Build history of the part. All positions in model axes, mm. Face numbers are marked on the shaded views. A direction names the side the tool comes from. Round coordinates to 2 decimals unless told otherwise and drop trailing zeros. Loops run counter-clockwise (first coordinate to the right, second up) from the corner with the lowest first, then second, coordinate; pieces in that order, holes last. Notation, with made-up numbers: (58, 23.5) - (80, 23.5) arc R4 cw to (80, 30.5) - close; hole circle Ø3 at (24, 23). An arc over 180 degrees is marked (long way). Use a Markdown table: item, result.
from build123d import *

# Parameters (mm, degrees)
BASE_BLOCK_SKETCH_W       = 90
BASE_BLOCK_SKETCH_H       = 45
BASE_BLOCK_90X45X60_DEPTH = 60
LUG_A_SKETCH_R            = 10
LUG_A_DEPTH               = 20
LUG_RECESS_CUT_DEPTH      = 5
LUG_B_DEPTH               = 20
LUG_HOLE_SKETCH_R         = 10
LUG_HOLES_DEPTH           = 114.357840488
ANGLED_SIDE_CUT_SKETCH_W  = 35
ANGLED_SIDE_CUT_SKETCH_H  = 40
ANGLED_SIDE_CUT_DEPTH     = 117.216392992
SIDE_BOSS_A_SKETCH_R      = 7.5
SIDE_BOSS_A_DEPTH         = 20
SIDE_BOSS_B_SKETCH_R      = 7.5
SIDE_BOSS_B_DEPTH         = 20
TOP_HOLE_SKETCH_R         = 12.5
TOP_HOLE_DEPTH            = 20
LUG_TOP_FILLET_R18_R      = 18
BOTTOM_SLOT_SKETCH_W      = 10
BOTTOM_SLOT_SKETCH_H      = 40
BOTTOM_SLOT_DEPTH         = 129.570019834


with BuildPart() as part:
    # Base Block Sketch → Base Block 90x45x60 (new body)
    with BuildSketch(Plane(origin=(0, 0, 0), x_dir=(1, 0, 0), z_dir=(0, 1, 0))):
        Rectangle(BASE_BLOCK_SKETCH_W, BASE_BLOCK_SKETCH_H)
    extrude(amount=-BASE_BLOCK_90X45X60_DEPTH)

    # Lug A Sketch → Lug A (add)
    with BuildSketch(Plane.XY.offset(22.5)):
        Polygon((-45, 0), (-45, -60), (45, -60), (45, 0), (0, 40), (-45, 40), align=None)
        with Locations((-8, 20)):
            Circle(LUG_A_SKETCH_R, mode=Mode.SUBTRACT)
    extrude(amount=LUG_A_DEPTH)

    # Lug Recess Sketch → Lug Recess Cut (cut)
    with BuildSketch(Plane(origin=(0, 0, 22.5), x_dir=(-1, 0, 0), z_dir=(0, 0, -1))):
        Polygon((-45, 0), (45, 0), (45, 40), (0, 40), align=None)
    extrude(amount=-LUG_RECESS_CUT_DEPTH, mode=Mode.SUBTRACT)

    # Lug B Sketch → Lug B (add)
    with BuildSketch(Plane(origin=(0, 0, -22.5), x_dir=(-1, 0, 0), z_dir=(0, 0, -1))):
        Polygon((-45, 0), (-45, -60), (45, -60), (45, 0), (45, 40), (0, 40), align=None)
    extrude(amount=LUG_B_DEPTH)

    # Lug Hole Sketch → Lug Holes (cut, through all)
    with BuildSketch(Plane.XY.offset(42.5)):
        with Locations((-8, 20)):
            Circle(LUG_HOLE_SKETCH_R)
    extrude(amount=-LUG_HOLES_DEPTH, mode=Mode.SUBTRACT)

    # Angled Side Cut Sketch → Angled Side Cut (cut, through all)
    with BuildSketch(Plane(origin=(45, 0, 0), x_dir=(0, 0, -1), z_dir=(1, 0, 0))):
        with Locations((-5, -40)):
            Rectangle(ANGLED_SIDE_CUT_SKETCH_W, ANGLED_SIDE_CUT_SKETCH_H)
    extrude(amount=-ANGLED_SIDE_CUT_DEPTH, mode=Mode.SUBTRACT)

    # Side Boss A Sketch → Side Boss A (add)
    with BuildSketch(Plane.ZY.offset(45)):
        with BuildLine():
            ThreePointArc((68.287962614, -7.064659931), (67.675104993, 4.552186853), (57.5, 10.190800338))
            Line((57.5, 10.190800338), (42.5, 10.190800338))
            Line((42.5, 10.190800338), (42.5, -60))
            Line((42.5, -60), (68.287962614, -7.064659931))
        make_face()
        with Locations((57.5, -1.809199662)):
            Circle(SIDE_BOSS_A_SKETCH_R, mode=Mode.SUBTRACT)
    extrude(amount=-SIDE_BOSS_A_DEPTH)

    # Side Boss B Sketch → Side Boss B (add)
    with BuildSketch(Plane.ZY.offset(45)):
        with BuildLine():
            Line((-42.5, 12), (-57.5, 12))
            ThreePointArc((-57.5, 12), (-67.633293922, 6.427779888), (-68.355763811, -5.113940953))
            Line((-68.355763811, -5.113940953), (-42.5, -60))
            Line((-42.5, -60), (-42.5, 12))
        make_face()
        with Locations((-57.5, 0)):
            Circle(SIDE_BOSS_B_SKETCH_R, mode=Mode.SUBTRACT)
    extrude(amount=-SIDE_BOSS_B_DEPTH)

    # Top Hole Sketch → Top Hole (cut)
    with BuildSketch(Plane(origin=(0, 0, 0), x_dir=(1, 0, 0), z_dir=(0, 1, 0))):
        with Locations(Location((30, -2.5, 0), (0, 0, 270))):
            Circle(TOP_HOLE_SKETCH_R)
    extrude(amount=-TOP_HOLE_DEPTH, mode=Mode.SUBTRACT)

    # Lug Top Fillet R18
    lug_top_fillet_r18_edges = [part.edges().sort_by_distance(p)[0] for p in [
        (0, 40, 35),
        (0, 40, -32.5),
    ]]
    fillet(lug_top_fillet_r18_edges, radius=LUG_TOP_FILLET_R18_R)

    # Bottom Slot Sketch → Bottom Slot (cut, through all)
    with BuildSketch(Plane(origin=(45, 0, 0), x_dir=(0, 0, -1), z_dir=(1, 0, 0))):
        with Locations((17.5, -40)):
            Rectangle(BOTTOM_SLOT_SKETCH_W, BOTTOM_SLOT_SKETCH_H)
    extrude(amount=-BOTTOM_SLOT_DEPTH, mode=Mode.SUBTRACT)


solid = part.part
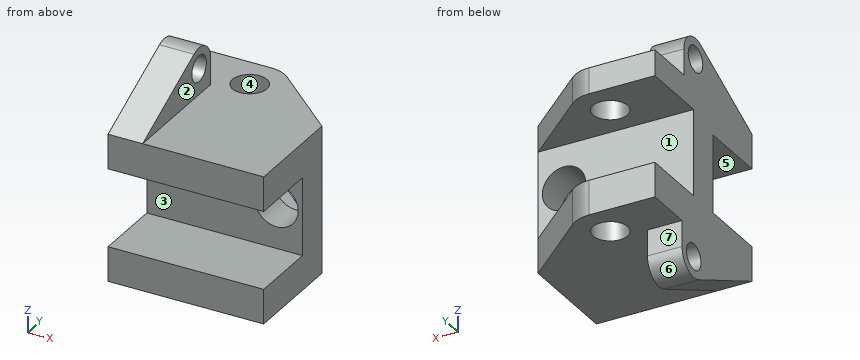
Q1. Cut at C-C, the plane x = 30. List the corners of the cut face in (y, z), plus the area to 3 significant figures.
Results found:
| item | result |
|---|---|
| outline | (-60, -42.5) - (13.33, -42.5) - (13.33, -22.5) - (0, -22.5) - (0, -10) - (-20, -10) - (-20, -22.5) - (-60, -22.5) - close; (-60, 22.5) - (-20, 22.5) - (-20, 15) - (0, 15) - (0, 27.5) - (13.33, 27.5) - (13.33, 42.5) - (-60, 42.5) - close |
| area | 3,270 mm2 |
Q2. Cut at A-A, the plane x = -16. List the corners of the cut face in (y, z), plus the area to 3 significant figures.
Results found:
| item | result |
|---|---|
| outline | (-60, -42.5) - (14, -42.5) - (14, -22.5) - (0, -22.5) - (0, 27.5) - (14, 27.5) - (14, 42.5) - (-60, 42.5) - (-60, 22.5) - (-20, 22.5) - (-20, -22.5) - (-60, -22.5) - close; (26, -42.5) - (40, -42.5) - (40, -22.5) - (26, -22.5) - close; (26, 27.5) - (40, 27.5) - (40, 42.5) - (26, 42.5) - close |
| area | 4,280 mm2 |
Q3. Cut at D-D, the plane y = -37. List the corners of the cut face in (x, z), plus the area to 3 significant figures.
Results found:
| item | result |
|---|---|
| outline | (-45, -53.33) - (-25, -53.33) - (-25, -42.5) - (45, -42.5) - (45, -22.5) - (-45, -22.5) - close; (-45, 22.5) - (45, 22.5) - (45, 42.5) - (-25, 42.5) - (-25, 53.7) - (-45, 53.7) - close |
| area | 4,040 mm2 |
Q4. Which spindle directions (+Z, -Z, +X, -X, +Y, -Y) get a long thin tool onto all of the face, cutting with end or side? Do the marked faces 1, 2, 3 and 4. Say none if no direction does.
Results found:
| item | result |
|---|---|
| face 1 | +X, -X, +Y |
| face 2 | +Z, +X, +Y, -Y |
| face 3 | +X, -X, -Y |
| face 4 | +Z, -Z |
Q5. Probe line 1 (Z direction, x = 7.5, y = -36); line 2 (Y direction, x = -8, z = 37.75); line 3 (Z direction, x = -28.5, y = -4). List the from-to ranges inside material, lowest first.
Results found:
| item | result |
|---|---|
| line 1 | z = -42.5 to -22.5, 22.5 to 42.5 |
| line 2 | y = -60 to 10, 30 to 40 |
| line 3 | z = -68.81 to -63.84, -51.16 to 50.33, 64.67 to 69.3 |
Q6. Drop flat-ended pins along their axis: pin 1 (15 mm diameter, centred on x = -14, z = 4, fed in from +Y); pin 2 (1.5 mm diameter, centred on x = -32.5, y = 17.5, fed in from -Z); pin 3 (2 mm diameter, centred on x = 10.5, z = -13.5, fed in from -Y); pin 4 (12 mm diameter, centred on y = -1.81, z = 57.5, fed in from +X). Give the stop position or say it passes through.
Results found:
| item | result |
|---|---|
| pin 1 | stops at y = 0 |
| pin 2 | stops at z = -42.5 |
| pin 3 | stops at y = -20 |
| pin 4 | passes through |
Q7. Pull direction Z, two halves, no side cores. Call the marked faces 5, 6 and 7: pulls with the +Z half, pulls with the -Z half, needs draft (parallel to the pull), parting line crosses it, or undercut.
Results found:
| item | result |
|---|---|
| face 5 | undercut |
| face 6 | pulls with the -Z half |
| face 7 | needs draft |
Q8. Cut at B-B, the plane z = 2.5. List the corners of the cut face in (x, y).
Results found:
| item | result |
|---|---|
| outline | (-45, -20) - (17.5, -20) - (17.5, 0) - (-45, 0) - close; (42.5, -20) - (45, -20) - (45, 0) - (42.5, 0) - close |
